```python
from build123d import *

# Parameters (mm, degrees)
SKETCH1_W                                          = 45
SKETCH1_H                                          = 110
BOSS_EXTRUDE1_DEPTH                                = 4
HOLE_SIZE_BASED_ON_SOCKET_HEAD_CAP_SCR_D           = 4.5
HOLE_SIZE_BASED_ON_SOCKET_HEAD_CAP_SCR_DEPTH       = 12.4
HOLE_SIZE_BASED_ON_SOCKET_HEAD_CAP_SCR_CBORE_D     = 8
HOLE_SIZE_BASED_ON_SOCKET_HEAD_CAP_SCR_CBORE_DEPTH = 4.6
HOLE_SIZE_BASED_ON_SOCKET_HEAD_CAP_SCR_TIP         = 1.351936393
SKETCH4_W                                          = 1
SKETCH4_H                                          = 10
CUT_EXTRUDE1_DEPTH                                 = 72.175838597
M3_TAPPED_HOLE1_D                                  = 2.5
CHAMFER1_SIZE                                      = 1
CUT_EXTRUDE2_DEPTH                                 = 60.960403601


with BuildPart() as part:
    # Sketch1 → Boss-Extrude1 (new, symmetric)
    with BuildSketch(Plane.XY):
        Rectangle(SKETCH1_W, SKETCH1_H)
    extrude(amount=BOSS_EXTRUDE1_DEPTH, both=True)

    # Hole size (% based on socket head cap screw type)1
    with Locations(Plane.XY.offset(4)):
        with Locations((-17.5, -50), (17.5, -50)):
            CounterBoreHole(HOLE_SIZE_BASED_ON_SOCKET_HEAD_CAP_SCR_D / 2, HOLE_SIZE_BASED_ON_SOCKET_HEAD_CAP_SCR_CBORE_D / 2, HOLE_SIZE_BASED_ON_SOCKET_HEAD_CAP_SCR_CBORE_DEPTH, depth=HOLE_SIZE_BASED_ON_SOCKET_HEAD_CAP_SCR_DEPTH)
            with Locations((0, 0, -(HOLE_SIZE_BASED_ON_SOCKET_HEAD_CAP_SCR_DEPTH + HOLE_SIZE_BASED_ON_SOCKET_HEAD_CAP_SCR_TIP / 2))):  # 118° drill point
                Cone(0, HOLE_SIZE_BASED_ON_SOCKET_HEAD_CAP_SCR_D / 2, HOLE_SIZE_BASED_ON_SOCKET_HEAD_CAP_SCR_TIP, mode=Mode.SUBTRACT)

    # Sketch4 → Cut-Extrude1 (cut, through all)
    with BuildSketch(Plane(origin=(22.5, 0, 0), x_dir=(0, 0, -1), z_dir=(1, 0, 0))):
        with Locations((3.5, -50)):
            Rectangle(SKETCH4_W, SKETCH4_H)
    extrude(amount=-CUT_EXTRUDE1_DEPTH, mode=Mode.SUBTRACT)

    # M3 Tapped Hole1 (through all)
    with Locations(Plane.XY.offset(4)):
        with Locations((0, 30), (0, 0)):
            Hole(M3_TAPPED_HOLE1_D / 2)

    # Chamfer1
    chamfer1_edges = [part.edges().sort_by_distance(p)[0] for p in [
        (22.5, -55, 0.5),
        (-22.5, -55, 0.5),
        (-22.5, 55, 0),
        (22.5, 55, 0),
    ]]
    chamfer(chamfer1_edges, length=CHAMFER1_SIZE)

    # Sketch7 → Cut-Extrude2 (cut, through all)
    with BuildSketch(Plane.XY.offset(4)):
        with BuildLine():
            Line((10, -10), (-10, -10))
            ThreePointArc((-10, -10), (-13.535533906, -11.464466094), (-15, -15))
            Line((-15, -15), (-15, -35))
            ThreePointArc((-15, -35), (-13.535533906, -38.535533906), (-10, -40))
            Line((-10, -40), (10, -40))
            ThreePointArc((10, -40), (13.535533906, -38.535533906), (15, -35))
            Line((15, -35), (15, -15))
            ThreePointArc((15, -15), (13.535533906, -11.464466094), (10, -10))
        make_face()
    extrude(amount=-CUT_EXTRUDE2_DEPTH, mode=Mode.SUBTRACT)


solid = part.part
```
CAD build for the part. Positions are in the model's coordinates, mm. A direction names the side the tool comes from. Round coordinates to 2 decimals unless told otherwise and drop trailing zeros. Loops run counter-clockwise (first coordinate to the right, second up) from the corner with the lowest first, then second, coordinate; pieces in that order, holes last. Notation, with made-up numbers: M -33.5,-9 L 2.5,-9 A19 cw 2.5,8 Z; hole C 73.5,3.25 d9. An arc over 180 degrees is marked long. Use a Markdown table: item, result. Add a question column.
(1) Cut at C-C (z = 1.5). Give the cut face in (x, y).
(2) Pull direction X, two halves, no side cores. Call faces 6 (the face through (-16, -52, -0.6)), 7 (the face through (22.5, -1, 0)), 8 (the face through (0, 55, 0)), 9 (the face through (-22.5, -1, 0)): +X half, -X half, draft (parallel to the pull), parting line (faces both ways), or undercut.
(3) Drill centre lines: line 1 (Y direction, x = 17.5, z = 2.6); line 2 (X direction, y = -24, z = 2.75); line 3 (Y direction, x = -6.5, z = 1.25). Where is each one in solid material? Low to high.
(4) Cut at A-A (x = -17.5). Give the cut face in (y, z), and give its area (3 significant figures).
(5) Cut at D-D (y = -24). Give the cut face in (x, z), and give its area (3 significant figures).
(6) Cut at B-B (y = 0). Give the cut face in (x, z).
(7) Flat gauge pins, fed straight in: pin 1 (1.1 mm diameter, centred on x = -10, z = -3.5, fed in from -Y); pin 2 (2.5 mm diameter, centred on x = -17.5, y = -50, fed in from +Z); pin 3 (6.5 mm diameter, centred on x = 17.5, y = -50, fed in from +Z); pin 4 (3 mm diameter, centred on x = -6.5, y = -47.5, fed in from -Z). Where does each tip first touch, or does it go through?
(8) Which spindle directions (+Z, -Z, +X, -X, +Y, -Y) get a long thin tool onto all of the face, cutting with end or side? Do faces 1 (the face through (0, 13, 4)), 2 (the face through (14.3, -52.4, 1.7)), 3 (the face through (0, -55, 1)), 4 (the face through (0, -50, -3)), 5 (the face through (-13, -11, 0)). Say none if no direction does.
Geometry says:
| question | item | result |
|---|---|---|
| 1 | outline | M -22.5,-54 L -21.5,-55 L 21.5,-55 L 22.5,-54 L 22.5,54 L 21.5,55 L -21.5,55 L -22.5,54 Z; hole C -17.5,-50 d8; hole M -15,-35 A5 ccw -10,-40 L 10,-40 A5 ccw 15,-35 L 15,-15 A5 ccw 10,-10 L -10,-10 A5 ccw -15,-15 Z; hole C 0,0 d2.5; hole C 0,30 d2.5; hole C 17.5,-50 d8 |
| 2 | face 6 | undercut |
| 2 | face 7 | +X half |
| 2 | face 8 | draft |
| 2 | face 9 | -X half |
| 3 | line 1 | y = -55 to -54, -46 to 55 |
| 3 | line 2 | x = -22.5 to -15, 15 to 22.5 |
| 3 | line 3 | y = -55 to -40, -10 to 55 |
| 4 | outline | M -55,-3 L -52.25,-3 L -52.25,-0.6 L -54,-0.6 L -54,4 L -55,4 Z; M -47.75,-3 L -45,-3 L -45,-4 L 55,-4 L 55,4 L -46,4 L -46,-0.6 L -47.75,-0.6 Z |
| 4 | area | 822 mm² |
| 5 | outline | M -22.5,-4 L -15,-4 L -15,4 L -22.5,4 Z; M 15,-4 L 22.5,-4 L 22.5,4 L 15,4 Z |
| 5 | area | 120 mm² |
| 6 | outline | M -22.5,-4 L -1.25,-4 L -1.25,4 L -22.5,4 Z; M 1.25,-4 L 22.5,-4 L 22.5,4 L 1.25,4 Z |
| 7 | pin 1 | stops at y = -55 |
| 7 | pin 2 | passes through |
| 7 | pin 3 | stops at z = -0.6 |
| 7 | pin 4 | stops at z = -3 |
| 8 | face 1 | +Z, +X, -X, +Y, -Y |
| 8 | face 2 | +Z |
| 8 | face 3 | +Z, -Z, +X, -X, -Y |
| 8 | face 4 | -Z, +X, -X, -Y |
| 8 | face 5 | +Z, -Z |
